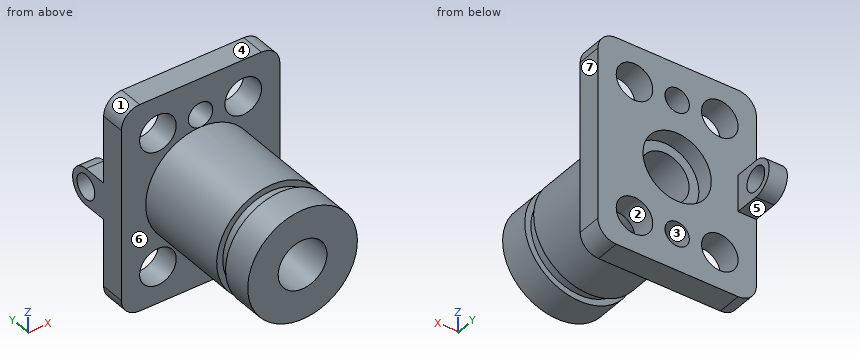
```python
from build123d import *

# Parameters (mm, degrees)
BARREL_SKETCH_R               = 45
HOUSING_BARREL_90_DEPTH       = 115
MOUNTING_FLANGE_SKETCH_W      = 130
MOUNTING_FLANGE_SKETCH_H      = 170
MOUNTING_FLANGE_170X130_DEPTH = 20
FLANGE_HOLES_SKETCH_R         = 15
FLANGE_HOLES_SKETCH_R_2       = 10
FLANGE_MOUNTING_HOLES_DEPTH   = 20
COUNTERBORE_SKETCH_R          = 28
COUNTERBORE_56_DEPTH          = 14
BORE_SKETCH_R                 = 20
BORE_40_DEPTH                 = 162.527087512
BARREL_GROOVE_SKETCH_W        = 45
BARREL_GROOVE_SKETCH_H        = 10
GROOVE_RING_SKETCH_W          = 40
GROOVE_RING_SKETCH_H          = 10
LIFTING_LUG_DEPTH             = 15
LUG_HOLE_SKETCH_R             = 10
LUG_HOLE_20_DEPTH             = 15
FLANGE_CORNER_FILLETS_R15_R   = 15
BOTTOM_RECESS_SKETCH_R        = 20
BOTTOM_RECESS_40_DEPTH        = 15


with BuildPart() as part:
    # Barrel Sketch → Housing Barrel Ø90 (new body)
    with BuildSketch(Plane(origin=(0, 0, 0), x_dir=(1, 0, 0), z_dir=(0, 1, 0))):
        with Locations(Location((0, 0, 0), (0, 0, 270))):
            Circle(BARREL_SKETCH_R)
    extrude(amount=HOUSING_BARREL_90_DEPTH)

    # Mounting Flange Sketch → Mounting Flange 170x130 (add)
    with BuildSketch(Plane(origin=(0, 115, 0), x_dir=(1, 0, 0), z_dir=(0, 1, 0))):
        Rectangle(MOUNTING_FLANGE_SKETCH_W, MOUNTING_FLANGE_SKETCH_H)
    extrude(amount=MOUNTING_FLANGE_170X130_DEPTH)

    # Flange Holes Sketch → Flange Mounting Holes (cut)
    with BuildSketch(Plane(origin=(0, 135, 0), x_dir=(1, 0, 0), z_dir=(0, 1, 0))):
        with Locations(Location((35, 55, 0), (0, 0, 270))):
            Circle(FLANGE_HOLES_SKETCH_R)
        with Locations(Location((0, 55, 0), (0, 0, 270))):
            Circle(FLANGE_HOLES_SKETCH_R_2)
        with Locations(Location((-35, 55, 0), (0, 0, 270))):
            Circle(FLANGE_HOLES_SKETCH_R)
        with Locations(Location((-35, -55, 0), (0, 0, 90))):
            Circle(FLANGE_HOLES_SKETCH_R)
        with Locations(Location((0, -55, 0), (0, 0, 89.999768226))):
            Circle(FLANGE_HOLES_SKETCH_R_2)
        with Locations(Location((35, -55, 0), (0, 0, 90))):
            Circle(FLANGE_HOLES_SKETCH_R)
    extrude(amount=-FLANGE_MOUNTING_HOLES_DEPTH, mode=Mode.SUBTRACT)

    # Counterbore Sketch → Counterbore Ø56 (cut)
    with BuildSketch(Plane(origin=(0, 135, 0), x_dir=(1, 0, 0), z_dir=(0, 1, 0))):
        with Locations(Location((0, 0, 0), (0, 0, 270))):
            Circle(COUNTERBORE_SKETCH_R)
    extrude(amount=-COUNTERBORE_56_DEPTH, mode=Mode.SUBTRACT)

    # Bore Sketch → Bore Ø40 (cut, through all)
    with BuildSketch(Plane(origin=(0, 121, 0), x_dir=(1, 0, 0), z_dir=(0, 1, 0))):
        with Locations(Location((0, 0, 0), (0, 0, 270))):
            Circle(BORE_SKETCH_R)
    extrude(amount=-BORE_40_DEPTH, mode=Mode.SUBTRACT)

    # Barrel Groove Sketch → Barrel Groove (revolve, cut)
    with BuildSketch(Plane.XY, mode=Mode.PRIVATE) as barrel_groove_sk:
        with Locations((-22.5, 30)):
            Rectangle(BARREL_GROOVE_SKETCH_W, BARREL_GROOVE_SKETCH_H)
    revolve(barrel_groove_sk.sketch.rotate(Axis((0, 25, 0), (0, 1, 0)), 90), axis=Axis((0, 25, 0), (0, 1, 0)), mode=Mode.SUBTRACT)


with BuildPart() as barrel_groove_piece_1:
    # of the separate pieces the step leaves, piece 1, a body of its own (barrel_groove_pieces)
    add(part.part.solids().sort_by_distance((-65, 115, 85))[0])



with BuildPart() as barrel_groove_piece_2:
    # of the separate pieces the step leaves, piece 2, a body of its own (barrel_groove_pieces)
    add(part.part.solids().sort_by_distance((0, 0, 45))[0])


with BuildPart() as barrel_groove_piece_1_1:
    add(barrel_groove_piece_1.part)

    add(barrel_groove_piece_2.part)  # Groove Ring merges Barrel Groove piece 2
    # Groove Ring Sketch → Groove Ring (revolve)
    with BuildSketch(Plane.XY, mode=Mode.PRIVATE) as groove_ring_sk:
        with Locations((-20, 30)):
            Rectangle(GROOVE_RING_SKETCH_W, GROOVE_RING_SKETCH_H)
    revolve(groove_ring_sk.sketch.rotate(Axis((0, 25, 0), (0, 1, 0)), 180), axis=Axis((0, 25, 0), (0, 1, 0)))

    # Lifting Lug Sketch → Lifting Lug (add)
    with BuildSketch(Plane.ZY.offset(65)):
        with BuildLine():
            Line((-15, 155), (-15, 135))
            Line((-15, 135), (15, 135))
            Line((15, 135), (15, 155))
            ThreePointArc((15, 155), (0, 170), (-15, 155))
        make_face()
    extrude(amount=-LIFTING_LUG_DEPTH)

    # Lug Hole Sketch → Lug Hole Ø20 (cut)
    with BuildSketch(Plane.ZY.offset(65)):
        with Locations((0, 155)):
            Circle(LUG_HOLE_SKETCH_R)
    extrude(amount=-LUG_HOLE_20_DEPTH, mode=Mode.SUBTRACT)

    # Flange Corner Fillets R15
    flange_corner_fillets_r15_edges = [barrel_groove_piece_1_1.edges().sort_by_distance(p)[0] for p in [
        (65, 125, 85),
        (65, 125, -85),
        (-65, 125, -85),
        (-65, 125, 85),
    ]]
    fillet(flange_corner_fillets_r15_edges, radius=FLANGE_CORNER_FILLETS_R15_R)

    # Bottom Recess Sketch → Bottom Recess Ø40 (cut)
    with BuildSketch(Plane.XZ.offset(-25)):
        with Locations(Location((0, 0, 0), (0, 0, 90))):
            Circle(BOTTOM_RECESS_SKETCH_R)
    extrude(amount=-BOTTOM_RECESS_40_DEPTH, mode=Mode.SUBTRACT)


solid = barrel_groove_piece_1_1.part
```
CAD build for the part. Positions are in the model's coordinates, mm. Face numbers are marked on the shaded views. A direction names the side the tool comes from. Round coordinates to 2 decimals unless told otherwise and drop trailing zeros. Write each loop counter-clockwise with the first axis right and the second up, starting at its lowest first coordinate (ties: lowest second). Pieces come first, ordered by that corner, then holes.
Item 1: Band-saw the part on D-D on x = -35. Write the cut outline in (y, z), then the cut area to 3 significant figures.
Filled in:
outline: (0, -28.28) - (25, -28.28) - (25, -19.36) - (35, -19.36) - (35, -28.28) - (115, -28.28) - (115, -40) - (135, -40) - (135, 40) - (115, 40) - (115, 28.28) - (35, 28.28) - (35, 19.36) - (25, 19.36) - (25, 28.28) - (0, 28.28) - close; (115, -85) - (135, -85) - (135, -70) - (115, -70) - close; (115, 70) - (135, 70) - (135, 85) - (115, 85) - close
area: 8,530 mm2
Item 2: Band-saw the part on A-A on z = 55. Write the cut outline in (x, y).
Filled in:
outline: (-65, 115) - (-50, 115) - (-50, 135) - (-65, 135) - close; (-20, 115) - (-10, 115) - (-10, 135) - (-20, 135) - close; (10, 115) - (20, 115) - (20, 135) - (10, 135) - close; (50, 115) - (65, 115) - (65, 135) - (50, 135) - close
Item 3: Drill centre lines: L1, parallel to X at y = 120.75, z = 55; L2, parallel to X at y = 125.25, z = 0; L3, parallel to Y at x = 42, z = 10.5. Where is each one in solid material? Low to high.
Filled in:
L1: x = -65 to -50, -20 to -10, 10 to 20, 50 to 65
L2: x = -65 to -28, 28 to 65
L3: y = 0 to 25, 35 to 135
Item 4: Mould opens along X. For the marked faces 1, 2, 3 and 4 say: released by +X, released by -X, zero draft, split by the parting line, or undercut.
Filled in:
face 1: released by -X
face 2: undercut
face 3: undercut
face 4: zero draft
Item 5: Band-saw the part on B-B on x = -7. Give the number of separate pieces and of enclosed holes in the cut face, then the cut area to 3 significant figures.
Filled in:
separate pieces: 4
enclosed holes: 0
area: 7,660 mm2
Item 6: Tool access for the marked faces 5, 6 and 7: list every direction of +Z, -Z, +X, -X, +Y, -Y with a clear straight run to the whole face (end or side of a thin tool).
Filled in:
face 5: -Z, +X, -X, +Y
face 6: -Y
face 7: +Z, -Z, +X, +Y, -Y
Item 7: Drop flat-ended pins along their axis: pin 1 Ø17 at (x, z) = (-12, 8) entering from +Y; pin 2 Ø4 at (x, y) = (-1.5, 79) entering from -Z; pin 3 Ø12 at (x, z) = (17.5, 34.5) entering from +Y. Give the stop position or say it passes through.
Filled in:
pin 1: stops at y = 121
pin 2: stops at z = -45
pin 3: stops at y = 135
